Design review of the part built by this model. Coordinates are the model's own, in mm. A direction names the side the tool comes from. Coordinates: 2 decimals unless noted, no trailing zeros. Write each loop counter-clockwise with the first axis right and the second up, starting at its lowest first coordinate (ties: lowest second). Pieces come first, ordered by that corner, then holes.
Q1. Take a section at C-C (y = -1.4). Give the boundary of the cut face in (x, z).
Q2. Take a section at B-B (x = 0). Give the boundary of the cut face in (y, z).
Q3. Insertion check: pin 1 (1 mm diameter, centred on x = 0.5, y = -0.5, fed in from +Z); pin 2 (1.5 mm diameter, centred on y = -2, z = 1, fed in from +X); pin 3 (3 mm diameter, centred on x = 0, z = -2, fed in from +Y). Each pin has a flat end and moves straight along its axis. Give the tip position at first contact, or say it passes through.
Q4. Take a section at A-A (z = 1). Give the boundary of the cut face in (x, y), and give its area (3 significant figures).
Q5. Mouldability with a two-part tool opening along X and no side actions: class faces 4 (the flat face through (1.113, 0.659, 1.26)), 5 (the flat face through (1.1, -1.1, 2)), 6 (the cylindrical face through (-1.5, 0.07, -2.96)) as pulls with the +X half, pulls with the -X half, needs draft (parallel to the pull), parting line crosses it, or undercut.
Q6. For probe 1 along Z at (x, y) = (-1.8, 1.3); probe 2 along Y at (x, z) = (0.55, 1); probe 3 along Y at (x, z) = (0, -2.25), list the stretches that pass through material, from the lowest coordinate up.
Q7. Machinability: for faces 1 (the flat face through (0, -2, 0)), 2 (the cylindrical face through (-0.54, -2.44, 0.99)), 3 (the flat face through (-1.13, 0.63, 1.26)), which of the approach directions +Z, -Z, +X, -X, +Y, -Y give a long, thin tool a straight path to every point of the face, cutting with its end or side? Answer none if there is none.
Q8. Take a section at D-D (z = -5). Give the boundary of the cut face in (x, y), and give its area (3 significant figures).
```python
from build123d import *

# Parameters (mm, degrees)
SKETCH1_R           = 1.5
BOSS_EXTRUDE1_DEPTH = 6
SKETCH2_R           = 2.5
BOSS_EXTRUDE2_DEPTH = 2
CUT_EXTRUDE1_DEPTH  = 1.5


with BuildPart() as part:
    # Sketch1 → Boss-Extrude1 (new body)
    with BuildSketch(Plane.XY):
        Circle(SKETCH1_R)
    extrude(amount=-BOSS_EXTRUDE1_DEPTH)

    # Sketch2 → Boss-Extrude2 (add)
    with BuildSketch(Plane.XY):
        Circle(SKETCH2_R)
    extrude(amount=BOSS_EXTRUDE2_DEPTH)

    # Sketch3 → Cut-Extrude1 (cut)
    with BuildSketch(Plane.XY.offset(2)):
        Polygon((0.722266578, 1.307190321), (-0.770926737, 1.279096365), (-1.493193314, -0.028093956), (-0.722266578, -1.307190321), (0.770926737, -1.279096365), (1.493193314, 0.028093956), align=None)
    extrude(amount=-CUT_EXTRUDE1_DEPTH, mode=Mode.SUBTRACT)


solid = part.part
```
Response:
1. outline: (-2.07, 0) - (-0.54, 0) - (-0.54, -6) - (0.54, -6) - (0.54, 0) - (2.07, 0) - (2.07, 2) - (-2.07, 2) - close
2. outline: (-2.5, 0) - (-1.5, 0) - (-1.5, -6) - (1.5, -6) - (1.5, 0) - (2.5, 0) - (2.5, 2) - (1.29, 2) - (1.29, 0.5) - (-1.29, 0.5) - (-1.29, 2) - (-2.5, 2) - close
3. pin 1: stops at z = 0.5
3. pin 2: stops at x = 2.17
3. pin 3: stops at y = 1.5
4. outline: circle Ø5 at (0, 0); hole (-1.49, -0.03) - (-0.72, -1.31) - (0.77, -1.28) - (1.49, 0.03) - (0.72, 1.31) - (-0.77, 1.28) - close
4. area: 13.8 mm2
5. face 4: undercut
5. face 5: needs draft
5. face 6: parting line crosses it
6. probe 1: z = 0 to 2
6. probe 2: y = -2.44 to -1.28, 1.3 to 2.44
6. probe 3: y = -1.5 to 1.5
7. face 1: -Z
7. face 2: +Z, -Z
7. face 3: +Z
8. outline: circle Ø3 at (0, 0)
8. area: 7.07 mm2
